```python
from build123d import *

# Parameters (mm, degrees)
SKETCH3_R          = 0.5
CUT_EXTRUDE1_DEPTH = 47.885498824
SKETCH4_OUTSIDE_W  = 28.164
SKETCH4_OUTSIDE_H  = 28.164
SKETCH4_OUTSIDE_R  = 1
CUT_EXTRUDE2_DEPTH = 3.5


with BuildPart() as part:
    # Sketch1 → Revolve1 (revolve)
    with BuildSketch(Plane.XY, mode=Mode.PRIVATE) as revolve1_sk:
        Polygon((0, 0), (1.5, 0), (1.5, 18.3), (8, 18.3), (8, 19), (3.75, 19), (3.75, 25.6), (1.5, 25.6), (1.5, 45.5), (0, 45.5), align=None)
    revolve(revolve1_sk.sketch.rotate(Axis((0, 0, 0), (0, 1, 0)), 90), axis=Axis((0, 0, 0), (0, 1, 0)))

    # Sketch3 → Cut-Extrude1 (cut, through all)
    with BuildSketch(Plane.XZ):
        with Locations(Location((0, 0, 0), (0, 0, 270))):
            Circle(SKETCH3_R)
    extrude(amount=-CUT_EXTRUDE1_DEPTH, mode=Mode.SUBTRACT)

    # Sketch4 outside → Cut-Extrude2 (cut)
    with BuildSketch(Plane(origin=(0, 45.5, 0), x_dir=(1, 0, 0), z_dir=(0, 1, 0))):
        Rectangle(SKETCH4_OUTSIDE_W, SKETCH4_OUTSIDE_H)
        with Locations(Location((0, 0, 0), (0, 0, 270))):
            Circle(SKETCH4_OUTSIDE_R, mode=Mode.SUBTRACT)
    extrude(amount=-CUT_EXTRUDE2_DEPTH, mode=Mode.SUBTRACT)


solid = part.part
```
Part model, mm, in its own coordinate system. A direction names the side the tool comes from. Round coordinates to 2 decimals unless told otherwise and drop trailing zeros. Loops run counter-clockwise (first coordinate to the right, second up) from the corner with the lowest first, then second, coordinate; pieces in that order, holes last.
1. Slice it at C-C (z = 2.5). Give the cut face in (x, y), and give its area (3 significant figures).
Solutions:
outline: (-7.6, 18.3) - (7.6, 18.3) - (7.6, 19) - (2.8, 19) - (2.8, 25.6) - (-2.8, 25.6) - (-2.8, 19) - (-7.6, 19) - close
area: 47.5 mm2
2. Slice it at B-B (y = 28). Give the cut face in (x, z).
Solutions:
outline: circle Ø3 at (0, 0); hole circle Ø1 at (0, 0)
3. Drill centre lines: line 1 along Y through (x, z) = (-2.5, -2.5); line 2 along Y through (x, z) = (1.25, 6.5); line 3 along X through (y, z) = (30, 0). Where is each one in solid material? Low to high.
Solutions:
line 1: y = 18.3 to 25.6
line 2: y = 18.3 to 19
line 3: x = -1.5 to -0.5, 0.5 to 1.5
4. Two-plate mould, pull along X, no slides. Class faces 1 (the face through (-1.89, 19, -3.44)), 2 (the face through (-0.488, 22.432, 0.108)), 3 (the face through (7.81, 18.65, 1.73)): pulls with the +X half, pulls with the -X half, needs draft (parallel to the pull), parting line crosses it, or undercut.
Solutions:
face 1: needs draft
face 2: undercut
face 3: parting line crosses it
5. 3-axis set-ups, long thin cutter, end or side, ignore diameter. For faces 4 (the face through (-0.45, 33.91, -1.43)), 5 (the face through (0, 0, 1)), 6 (the face through (-0.45, 9.28, -1.43)): which of +Z, -Z, +X, -X, +Y, -Y reach the whole face in a straight line?
Solutions:
face 4: +Y
face 5: +Z, -Z, +X, -X, -Y
face 6: -Y
6. Flat gauge pins, fed straight in: pin 1 (1 mm diameter, centred on x = -4.5, z = 1, fed in from +Y); pin 2 (5 mm diameter, centred on x = 6, z = -4, fed in from -Y); pin 3 (8 mm diameter, centred on y = 10.5, z = -3, fed in from -X). Where does each tip first touch, or does it go through?
Solutions:
pin 1: stops at y = 19
pin 2: stops at y = 18.3
pin 3: stops at x = -1.5
7. Slice it at A-A (z = 0). Give the cut face in (x, y), and give its area (3 significant figures).
Solutions:
outline: (-8, 18.3) - (-1.5, 18.3) - (-1.5, 0) - (-0.5, 0) - (-0.5, 45.5) - (-1, 45.5) - (-1, 42) - (-1.5, 42) - (-1.5, 25.6) - (-3.75, 25.6) - (-3.75, 19) - (-8, 19) - close; (0.5, 0) - (1.5, 0) - (1.5, 18.3) - (8, 18.3) - (8, 19) - (3.75, 19) - (3.75, 25.6) - (1.5, 25.6) - (1.5, 42) - (1, 42) - (1, 45.5) - (0.5, 45.5) - close
area: 126 mm2
8. Slice it at D-D (x = 4.25). Give the cut face in (y, z).
Solutions:
outline: (18.3, -6.78) - (19, -6.78) - (19, 6.78) - (18.3, 6.78) - close
